from build123d import *

# Parameters (mm, degrees)
HUB_BODY_REVOLVE_270DEG_ANGLE = 270


with BuildPart() as part:
    # Hub Profile Sketch → Hub Body Revolve 270deg (revolve)
    with BuildSketch(Plane(origin=(0, 0, 0), x_dir=(0, 0, -1), z_dir=(1, 0, 0))):
        Polygon((0, 0), (0, 27), (34, 40), (50, 40), (50, 50), (70, 50), (70, 32.5), (100, 32.5), (100, 0), align=None)
    revolve(axis=Axis((0, 0, -100), (0, 0, 1)), revolution_arc=HUB_BODY_REVOLVE_270DEG_ANGLE)

    # Tapered Bore Profile Sketch → Stepped Tapered Bore Cut (revolve, cut)
    with BuildSketch(Plane(origin=(0, 0, 0), x_dir=(0, 0, -1), z_dir=(1, 0, 0))):
        Polygon((0, 0), (0, 17), (34, 15.380026541), (34, 12), (47.09584733, 12), (100, 26.175624984), (100, 0), align=None)
    revolve(axis=Axis((0, 0, 0), (0, 0, -1)), mode=Mode.SUBTRACT)


solid = part.part
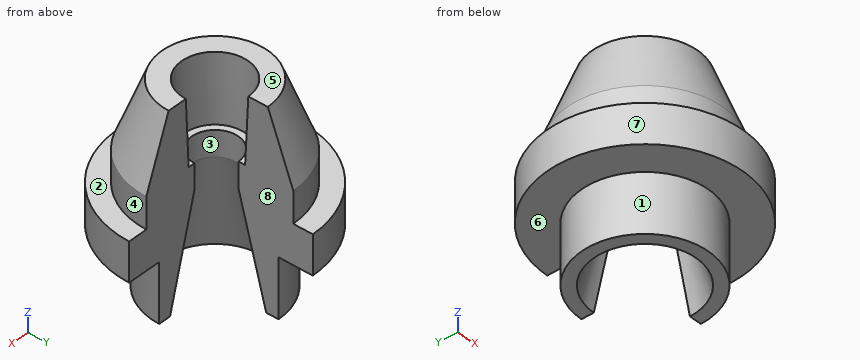
Could you check a few things on this model? Use its own coordinates, in mm. Face numbers are marked on the shaded views. A direction names the side the tool comes from. Round coordinates to 2 decimals unless told otherwise and drop trailing zeros. Loops run counter-clockwise (first coordinate to the right, second up) from the corner with the lowest first, then second, coordinate; pieces in that order, holes last. Notation, with made-up numbers: (57, 8) -> (74, 8) arc R25 ccw to (74, 41) -> close; hole circle Ø10 at (51, 11.5). An arc over 180 degrees is marked (long way). Use CSV: the item, a comma, the result in double quotes.
(1) If I drill on probe 1 along Z at (x, y) = (-11.5, -45.5); probe 2 along X at (y, z) = (-19.5, -81.5); probe 3 along X at (y, z) = (-38, -59.5), over which ranges is the centre line in solid material (lowest first)? Write a range as [from, to].
Return value:
probe 1,"z = [-70, -50]"
probe 2,"x = [-26, -8.37], [8.37, 26]"
probe 3,"x = [-32.5, 32.5]"
(2) Will these pins go through, and if not, where does the flat tip stop? pin 1 Ø1.5 at (y, z) = (29.5, -15) entering from -X; pin 2 Ø1 at (y, z) = (1, -51) entering from -X; pin 3 Ø6 at (y, z) = (-15, -85) entering from +X; pin 4 Ø5 at (x, y) = (-4.5, 21.5) entering from +Z.
Return value:
pin 1,"stops at x = -15.78"
pin 2,"stops at x = -50"
pin 3,"stops at x = 30.2"
pin 4,"stops at z = 0"
(3) For the marked faces 4, 5, 6, 7 and 8, which set-ups out of +Z, -Z, +X, -X, +Y, -Y let a thin tool reach every point of the face, with its end or its side?
Return value:
face 4,"+Z"
face 5,"+Z, +X, -X, +Y, -Y"
face 6,"-Z"
face 7,"+Z, -Z"
face 8,"+Z, -Z, +X, +Y"
(4) Suppose I cut it at B-B on z = -88.5. Write out the boundary of the cut face in (x, y), plus the area to 3 significant figures.
Return value:
outline,"(0, 23.09) -> (0, 32.5) arc R32.5 ccw (long way) to (32.5, 0) -> (23.09, 0) arc R23.09 cw (long way) to start"
area,"1,230 mm²"
(5) If we mould it in two halves opening along Y, with no side actions, what happens to the marked faces 1, 2 and 3? For each: +Y half, -Y half, draft (parallel to the pull), parting line (faces both ways), or undercut.
Return value:
face 1,"parting line"
face 2,"draft"
face 3,"undercut"
(6) Suppose I cut it at A-A on z = -77. Write out the boundary of the cut face in (x, y).
Return value:
outline,"(0, 20.01) -> (0, 32.5) arc R32.5 ccw (long way) to (32.5, 0) -> (20.01, 0) arc R20.01 cw (long way) to start"
